from build123d import *

# Parameters (mm, degrees)
SKETCH_1_R          = 37.5
SKETCH_1_R_2        = 11
EXTRUDE_1_DEPTH     = 5
SKETCH_2_R          = 23.5
SKETCH_2_R_2        = 21.5
EXTRUDE_2_DEPTH     = 5
SKETCH_3_R          = 3
CUT_EXTRUDE_1_DEPTH = 54.967582862
CHAMFER_1_SIZE      = 0.5
FILLET_1_R          = 1
CHAMFER_2_SIZE      = 0.5


with BuildPart() as part:
    # 草图1 → 拉伸1 (new body)
    with BuildSketch(Plane(origin=(0, 0, 0), x_dir=(1, 0, 0), z_dir=(0, 1, 0))):
        with Locations(Location((0, 0, 0), (0, 0, 270))):
            Circle(SKETCH_1_R)
        with Locations(Location((0, 0, 0), (0, 0, 270))):
            Circle(SKETCH_1_R_2, mode=Mode.SUBTRACT)
    extrude(amount=EXTRUDE_1_DEPTH)

    # 草图2 → 拉伸2 (add)
    with BuildSketch(Plane.XZ):
        with Locations(Location((0, 0, 0), (0, 0, 90))):
            Circle(SKETCH_2_R)
        with Locations(Location((0, 0, 0), (0, 0, 270))):
            Circle(SKETCH_2_R_2, mode=Mode.SUBTRACT)
    extrude(amount=EXTRUDE_2_DEPTH)

    # 草图3 → 切除-拉伸1 (cut, through all)
    with BuildSketch(Plane(origin=(0, 5, 0), x_dir=(-1, 0, 0), z_dir=(0, 1, 0))):
        with Locations(Location((-30, 0, 0), (0, 0, 90))):
            Circle(SKETCH_3_R)
        with Locations(Location((0, 30, 0), (0, 0, 90))):
            Circle(SKETCH_3_R)
        with Locations(Location((30, 0, 0), (0, 0, 90))):
            Circle(SKETCH_3_R)
        with Locations(Location((0, -30, 0), (0, 0, 90))):
            Circle(SKETCH_3_R)
    extrude(amount=-CUT_EXTRUDE_1_DEPTH, mode=Mode.SUBTRACT)

    # 倒角1
    chamfer_1_edges = [part.edges().sort_by_distance(p)[0] for p in [
        (0, -5, -23.5),
        (0, -5, 21.5),
        (0, 0, -37.5),
        (0, 5, -37.5),
    ]]
    chamfer(chamfer_1_edges, length=CHAMFER_1_SIZE)

    # 圆角1
    fillet_1_edges = [part.edges().sort_by_distance(p)[0] for p in [
        (0, 0, 21.5),
    ]]
    fillet(fillet_1_edges, radius=FILLET_1_R)

    # 倒角2
    chamfer_2_edges = [part.edges().sort_by_distance(p)[0] for p in [
        (0, 0, -11),
        (0, 5, -11),
    ]]
    chamfer(chamfer_2_edges, length=CHAMFER_2_SIZE)


solid = part.part
Read the model definition and answer for the solid it produces. Units are mm, in the model's axes. A direction names the side the tool comes from. Coordinates: 2 decimals unless noted, no trailing zeros. Write each loop counter-clockwise with the first axis right and the second up, starting at its lowest first coordinate (ties: lowest second). Pieces come first, ordered by that corner, then holes. Notation, with made-up numbers: M -15,-19.5 L 18,-19.5 A6 cw 18,-14.5 Z; hole C 53,40.5 d4. An arc over 180 degrees is marked long. Use a Markdown table: item, result.
Q1. Each of these flat-tipped pins is pushed along its axis until it touches: pin 1 Ø4 at (x, y) = (17, -3.5) entering from +Z; pin 2 Ø6 at (x, y) = (5, 2.5) entering from -Z; pin 3 Ø1 at (x, y) = (18.5, 3.5) entering from +Z. Where does it stop, or does it pass through?
Answer block:
| item | result |
|---|---|
| pin 1 | stops at z = 18.09 |
| pin 2 | stops at z = -37.45 |
| pin 3 | stops at z = 32.9 |
Q2. The part is cut by section B-B, the plane y = -2.75. Write down the section's boundary in (x, z).
Answer block:
| item | result |
|---|---|
| outline | C 0,0 d47; hole C 0,0 d43 |
Q3. Straight lines are drawn through the part: L1, parallel to X at y = 3.15, z = 0; L2, parallel to X at y = 4, z = -1.5; L3, parallel to Y at x = -20, z = -0.5. For each, find the intervals that lie inside material, in ascending order. Write a range as [from, to].
Answer block:
| item | result |
|---|---|
| L1 | x = [-37.5, -33], [-27, -11], [11, 27], [33, 37.5] |
| L2 | x = [-37.47, -32.6], [-27.4, -10.9], [10.9, 27.4], [32.6, 37.47] |
| L3 | y = [0, 5] |
Q4. The part is cut by section A-A, the plane z = 0. Give the number of separate pieces and of enclosed holes in the cut face, then the cut area to 3 significant figures.
Answer block:
| item | result |
|---|---|
| separate pieces | 4 |
| enclosed holes | 0 |
| area | 224 mm2 |
Q5. Which of the six approach directions +Z, -Z, +X, -X, +Y, -Y give full straight-line access (tool end or side, diameter ignored) to faces 1 (the face through (-9, 0, 9)), 2 (the face through (9, 5, 8))?
Answer block:
| item | result |
|---|---|
| face 1 | -Y |
| face 2 | +Z, -Z, +X, -X, +Y |
